CAD build for the part. Positions are in the model's coordinates, mm. Face numbers are marked on the shaded views. A direction names the side the tool comes from. Round coordinates to 2 decimals unless told otherwise and drop trailing zeros. Write each loop counter-clockwise with the first axis right and the second up, starting at its lowest first coordinate (ties: lowest second). Pieces come first, ordered by that corner, then holes. Notation, with made-up numbers: (76, 56.25) - (95, 56.25) arc R13 ccw to (95, 76.25) - close; hole circle Ø5 at (-39.5, 64.25). An arc over 180 degrees is marked (long way). Use one line per item in the form item = value. Start each with the question number.
Item 1: Band-saw the part on A-A, the plane x = 3.5. List the corners of the cut face in (y, z), and give its area (3 significant figures).
Item 2: Drill centre lines: L1, parallel to Y at x = 11, z = -1; L2, parallel to Z at x = 1, y = 1.5; L3, parallel to Y at x = 5, z = -0.1. Where is each one in solid material? Low to high.
Item 3: Pin check, flat tip, straight feed: pin 1 (1.5 mm diameter, centred on y = -1.5, z = 0.5, fed in from +X). Stop position of the tip, or through.
Item 4: Tool access for the marked faces 1 and 2: list every direction of +Z, -Z, +X, -X, +Y, -Y with a clear straight run to the whole face (end or side of a thin tool).
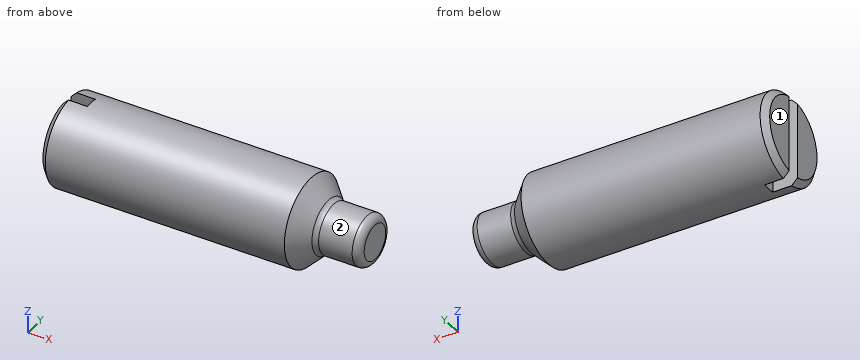
from build123d import *

# Parameters (mm, degrees)
SKETCH4_W          = 1.12
SKETCH4_H          = 0.6
CUT_EXTRUDE1_DEPTH = 50
FILLET1_R          = 0.3375


with BuildPart() as part:
    # Sketch3 → Base-Revolve (revolve)
    with BuildSketch(Plane.XY, mode=Mode.PRIVATE) as base_revolve_sk:
        Polygon((0, 0), (0, 1.732), (0.268, 2), (11.125, 2), (12, 1.125), (14, 1.125), (14, 0), align=None)
    revolve(base_revolve_sk.sketch.rotate(Axis((0, 0, 0), (1, 0, 0)), 90), axis=Axis((0, 0, 0), (1, 0, 0)))

    # Sketch4 → Cut-Extrude1 (cut, symmetric)
    with BuildSketch(Plane.XY):
        with Locations((0.56, 0)):
            Rectangle(SKETCH4_W, SKETCH4_H)
    extrude(amount=CUT_EXTRUDE1_DEPTH, both=True, mode=Mode.SUBTRACT)

    # Fillet1
    fillet1_edges = [part.edges().sort_by_distance(p)[0] for p in [
        (14, 0, -1.125),
        (12, 0, -1.125),
    ]]
    fillet(fillet1_edges, radius=FILLET1_R)


solid = part.part
Determined:
q1.outline = circle Ø4 at (0, 0)
q1.area = 12.6 mm²
q2.L1 = -1.73 to 1.73
q2.L2 = -1.32 to 1.32
q2.L3 = -2 to 2
q3.pin_1 = 14
q4.face_1 = +Z, -Z, -X, +Y, -Y
q4.face_2 = +X
